For this review, take the finished solid that the model builds, in its own axes (mm). Round coordinates to 2 decimals unless told otherwise and drop trailing zeros. Loops run counter-clockwise (first coordinate to the right, second up) from the corner with the lowest first, then second, coordinate; pieces in that order, holes last.
1) Take a section at A-A (z = 817). State the section outline as (x, y) points.
2) Take a section at B-B (x = 40). State the section outline as (y, z) points.
3) Take a section at C-C (y = 46.5). State the section outline as (x, z) points, then the cut area to 3 significant figures.
4) Insertion check: pin 1 (0.9 mm diameter, centred on x = 124.5, z = 833, fed in from -Y); pin 2 (6.5 mm diameter, centred on y = 20, z = 121, fed in from -X); pin 3 (8 mm diameter, centred on x = 28, z = 1188.5, fed in from -Y); pin 4 (13 mm diameter, centred on y = 80, z = 527, fed in from +X). Each pin has a flat end and moves straight along its axis. Give the tip position at first contact, or say it passes through.
5) Wall thickness on L1, parallel to X at y = 119, z = 1172; L2, parallel to Y at x = 1.7, z = 121; L3, parallel to Y at x = 1.25, z = 1339: over which ranges is each line inside the solid? List them lowest first.
6) Mouldability with a two-part tool opening along X and no side actions: class faces 1 (the flat face through (64, 127, 720)), 2 (the flat face through (0, 62, 720)), 3 (the flat face through (62, 130, 720)) as pulls with the +X half, pulls with the -X half, needs draft (parallel to the pull), parting line crosses it, or undercut.
```python
from build123d import *

# Parameters (mm, degrees)
BOSS_EXTRUDE1_DEPTH = 1460
SKETCH2_R           = 4
CUT_EXTRUDE1_DEPTH  = 1460


with BuildPart() as part:
    # Sketch1 → Boss-Extrude1 (new body)
    with BuildSketch(Plane.XY):
        with BuildLine():
            Line((0, 0), (0, 125))
            ThreePointArc((0, 125), (1.464466094, 128.535533906), (5, 130))
            Line((5, 130), (121, 130))
            ThreePointArc((121, 130), (124.535533906, 128.535533906), (126, 125))
            Line((126, 125), (126, 110))
            Line((126, 110), (123, 110))
            Line((123, 110), (123, 125))
            ThreePointArc((123, 125), (122.414213562, 126.414213562), (121, 127))
            Line((121, 127), (5, 127))
            ThreePointArc((5, 127), (3.585786438, 126.414213562), (3, 125))
            Line((3, 125), (3, 0))
            Line((3, 0), (0, 0))
        make_face()
    extrude(amount=BOSS_EXTRUDE1_DEPTH)

    # Sketch2 → Cut-Extrude1 (cut)
    with BuildSketch(Plane.ZY):
        with Locations((121, 80)):
            Circle(SKETCH2_R)
        with Locations((1339, 80)):
            Circle(SKETCH2_R)
        with Locations((933, 80)):
            Circle(SKETCH2_R)
        with Locations((527, 80)):
            Circle(SKETCH2_R)
        with Locations((121, 20)):
            Circle(SKETCH2_R)
        with Locations((1339, 20)):
            Circle(SKETCH2_R)
        with Locations((933, 20)):
            Circle(SKETCH2_R)
        with Locations((527, 20)):
            Circle(SKETCH2_R)
    extrude(amount=-CUT_EXTRUDE1_DEPTH, mode=Mode.SUBTRACT)


solid = part.part
```
Response:
1. outline: (0, 0) - (3, 0) - (3, 125) arc R2 cw to (5, 127) - (121, 127) arc R2 cw to (123, 125) - (123, 110) - (126, 110) - (126, 125) arc R5 ccw to (121, 130) - (5, 130) arc R5 ccw to (0, 125) - close
2. outline: (127, 0) - (130, 0) - (130, 1460) - (127, 1460) - close
3. outline: (0, 0) - (3, 0) - (3, 1460) - (0, 1460) - close
3. area: 4,380 mm2
4. pin 1: stops at y = 110
4. pin 2: passes through
4. pin 3: stops at y = 127
4. pin 4: stops at x = 3
5. L1: x = 0 to 3, 123 to 126
5. L2: y = 0 to 16, 24 to 76, 84 to 128.76
5. L3: y = 0 to 16, 24 to 76, 84 to 128.31
6. face 1: undercut
6. face 2: pulls with the -X half
6. face 3: needs draft
